Part model, mm, in its own coordinate system. Round coordinates to 2 decimals unless told otherwise and drop trailing zeros. Write each loop counter-clockwise with the first axis right and the second up, starting at its lowest first coordinate (ties: lowest second). Pieces come first, ordered by that corner, then holes.
```python
from build123d import *

# Parameters (mm, degrees)
SKETCH1_R               = 465
SKETCH1_R_2             = 390
BOSS_EXTRUDE1_DEPTH     = 45
M24_THREADED_HOLE1_D    = 21
CIRCULAR_PATTERN1_COUNT = 24


with BuildPart() as part:
    # Sketch1 → Boss-Extrude1 (new body)
    with BuildSketch(Plane.XY):
        with Locations(Location((0, 0, 0), (0, 0, 180))):
            Circle(SKETCH1_R)
        with Locations(Location((0, 0, 0), (0, 0, 180))):
            Circle(SKETCH1_R_2, mode=Mode.SUBTRACT)
    extrude(amount=BOSS_EXTRUDE1_DEPTH)

    # M24 Threaded hole1 (through all)
    with Locations(Plane(origin=(-422, 0, 45), x_dir=(1, 0, 0), z_dir=(0, 0, 1))):
        with Locations((0, 0)):
            m24_threaded_hole1 = Hole(M24_THREADED_HOLE1_D / 2)

    # Circular pattern1: M24 Threaded hole1 ×24 about axis
    circular_pattern1_axis = Axis((0, 0, 0), (0, 0, 1))
    for i in range(1, CIRCULAR_PATTERN1_COUNT):
        add(m24_threaded_hole1.rotate(circular_pattern1_axis, i * 360 / CIRCULAR_PATTERN1_COUNT), mode=Mode.SUBTRACT)


solid = part.part
```
Q1. Cut at C-C on z = 12. State how many separate pieces and enclosed holes the cut face has, plus the area to 3 significant figures.
Values follow:
separate pieces: 1
enclosed holes: 25
area: 193,000 mm2
Q2. Cut at B-B on x = 171. Write the cut outline in (y, z), plus the area to 3 significant figures.
Values follow:
outline: (-432.42, 0) - (-350.51, 0) - (-350.51, 45) - (-432.42, 45) - close; (350.51, 0) - (432.42, 0) - (432.42, 45) - (350.51, 45) - close
area: 7,370 mm2
Q3. Wall check: L1, parallel to X at y = -0.5, z = 11; L2, parallel to Y at x = 300, z = 23.5; L3, parallel to X at y = -295, z = 5.5. Give the ranges that are in metal, low to high.
Values follow:
L1: x = -465 to -432.49, -411.51 to -390, 390 to 411.51, 432.49 to 465
L2: y = -355.28 to -308.78, -288.02 to -249.2, 249.2 to 288.02, 308.78 to 355.28
L3: x = -359.44 to -308.33, -288.46 to -255.1, 255.1 to 288.46, 308.33 to 359.44
Q4. Drop flat-ended pins along their axis: pin 1 (10 mm diameter, centred on y = 146.5, z = 31, fed in from -X); pin 2 (24 mm diameter, centred on x = 0, y = -422, fed in from +Z); pin 3 (6 mm diameter, centred on y = 175, z = 7.5, fed in from -X); pin 4 (10 mm diameter, centred on y = -238, z = 8.5, fed in from -X). Give the stop position or say it passes through.
Values follow:
pin 1: stops at x = -442.95
pin 2: stops at z = 45
pin 3: stops at x = -432.02
pin 4: stops at x = -402.41
Q5. Cut at A-A on y = -23. Write the cut outline in (x, z).
Values follow:
outline: (-464.43, 0) - (-389.32, 0) - (-389.32, 45) - (-464.43, 45) - close; (389.32, 0) - (464.43, 0) - (464.43, 45) - (389.32, 45) - close
Q6. Mould opens along X. For faces 1 (the cylindrical face through (100.803, 453.942, 22.185)), 2 (the flat face through (-101, -381, 0)), 3 (the cylindrical face through (-201.3, 369.48, 22.18)) say: +X half, -X half, draft (parallel to the pull), parting line (faces both ways), or undercut.
Values follow:
face 1: parting line
face 2: draft
face 3: undercut
